from build123d import *

# Parameters (mm, degrees)
BASE_PLATE_SKETCH_W      = 78
BASE_PLATE_SKETCH_H      = 28
BASE_PLATE_78X28X8_DEPTH = 8
STEP_BLOCK_DEPTH         = 18
V_NOTCH_UPRIGHT_REACH    = 60.83


with BuildPart() as part:
    # Base Plate Sketch → Base Plate 78x28x8 (new body)
    with BuildSketch(Plane(origin=(0, 0, 0), x_dir=(1, 0, 0), z_dir=(0, 1, 0))):
        Rectangle(BASE_PLATE_SKETCH_W, BASE_PLATE_SKETCH_H)
    extrude(amount=BASE_PLATE_78X28X8_DEPTH)

    # Step Block Sketch → Step Block (add)
    with BuildSketch(Plane(origin=(0, 0, -14), x_dir=(-1, 0, 0), z_dir=(0, 0, -1))):
        Polygon((39, 8), (39, 16), (15, 16), (15, 34), (-1, 34), (-1, 8), align=None)
    extrude(amount=-STEP_BLOCK_DEPTH)

    # V-Notch Upright: up to this face of the body (flat: up to its plane)
    v_notch_upright_end = Plane(part.part.faces().sort_by_distance((-6.571428571, 10.987012987, -14))[0])
    # V-Notch Upright Sketch → V-Notch Upright (add, up to the picked face)
    with BuildSketch(Plane.XY.offset(14), mode=Mode.PRIVATE) as v_notch_upright_sk1:
        Polygon((-11.123999112, 8), (12.191383796, 58), (25.786000601, 51.660726074), (10.571743179, 19.033645741), (15.103282114, 16.920554432), (30.317539536, 49.547634765), (39, 45.498936959), (39, 8), align=None)
    v_notch_upright_tool1 = split(extrude(v_notch_upright_sk1.sketch, amount=-V_NOTCH_UPRIGHT_REACH, mode=Mode.PRIVATE), bisect_by=v_notch_upright_end, keep=Keep.BOTH, mode=Mode.PRIVATE)
    add(v_notch_upright_tool1.solids().sort_by(Axis((1.175344, 32.700793, 14), (0, 0, -1)))[0])


solid = part.part
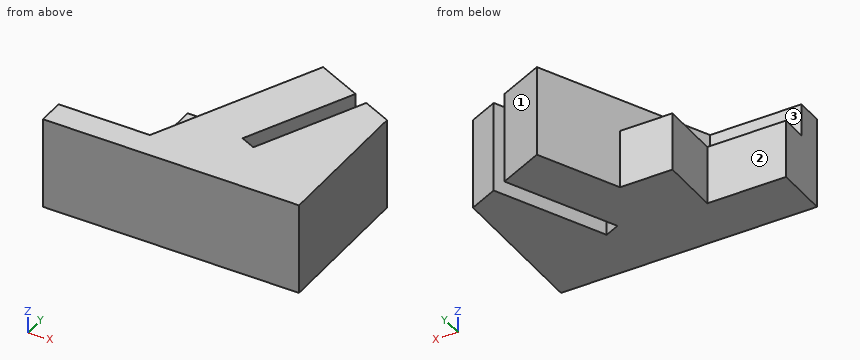
Check sheet for the modelled part. Datum: model origin and axes. Units: mm. Face numbers are marked on the shaded views. A direction names the side the tool comes from. Round coordinates to 2 decimals unless told otherwise and drop trailing zeros. Write each loop counter-clockwise with the first axis right and the second up, starting at its lowest first coordinate (ties: lowest second). Pieces come first, ordered by that corner, then holes. Notation, with made-up numbers: (-20, -28) - (34, -28) arc R16 cw to (34, -21) - close; hole circle Ø3 at (87.25, -13). An arc over 180 degrees is marked (long way). Return JSON: item names as keys, results as strings.
Q1. Cross-section at D-D (y = 44). Record the boundary of the cut face in (x, z).
Returned:
{"outline": "(5.66, -14) - (22.21, -14) - (22.21, 14) - (5.66, 14) - close; (27.73, -14) - (39, -14) - (39, 14) - (27.73, 14) - close"}
Q2. Cross-section at B-B (y = 18). Record the boundary of the cut face in (x, z), then the cut area to 3 significant figures.
Returned:
{"outline": "(-15, -14) - (12.79, -14) - (12.79, 14) - (-6.46, 14) - (-6.46, 4) - (-15, 4) - close; (15.61, -14) - (39, -14) - (39, 14) - (15.61, 14) - close", "area": "1,350 mm²"}
Q3. Cross-section at C-C (z = 7). Record the boundary of the cut face in (x, y), then the cut area to 3 significant figures.
Returned:
{"outline": "(-39, 0) - (39, 0) - (39, 45.5) - (30.32, 49.55) - (15.1, 16.92) - (10.57, 19.03) - (25.79, 51.66) - (12.19, 58) - (-11.12, 8) - (-39, 8) - close", "area": "2,200 mm²"}
Q4. Cross-section at A-A (x = 23). Record the boundary of the cut face in (y, z), then the cut area to 3 significant figures.
Returned:
{"outline": "(0, -14) - (33.86, -14) - (33.86, 14) - (0, 14) - close; (45.69, -14) - (52.96, -14) - (52.96, 14) - (45.69, 14) - close", "area": "1,150 mm²"}
Q5. Access from +Z, -Z, +X, -X, +Y, -Y to the whole of each face (thin tool, end or side, straight path). Record for the marked faces 1, 2 and 3.
Returned:
{"face 1": "+Z, -Z, +X, +Y", "face 2": "+Z, -Z, -X, +Y", "face 3": "+Z, -X, +Y"}
Q6. Scan lines: L1, parallel to Y at x = -15, z = 7.25; L2, parallel to Y at x = -33, z = -3; L3, parallel to X at y = 19, z = -1.75. Record each from-to range of solid material in increasing order. Write a range as from..to.
Returned:
{"L1": "y = 0..8", "L2": "y = 0..16", "L3": "x = -15..10.64, 16.07..39"}
Q7. Depth check by flat-ended pin: P1, Ø2, axis at y = 12.5, z = 9.5, coming from the -X side; P2, Ø9, axis at y = 28.5, z = -4, coming from the -X side; P3, Ø5.5, axis at x = -29.5, z = -6.5, coming from the +Y side. Enter the tip coordinate at first touch or a pass-through.
Returned:
{"P1": "stops at x = -9.49", "P2": "stops at x = -15", "P3": "stops at y = 16"}
